The drawing under review shows one solid part. Ordinate dimensions are in mm from its lowest x, y, z. Coordinates: 2 decimals unless noted, no trailing zeros. Loops run counter-clockwise (first coordinate to the right, second up) from the corner with the lowest first, then second, coordinate; pieces in that order, holes last.
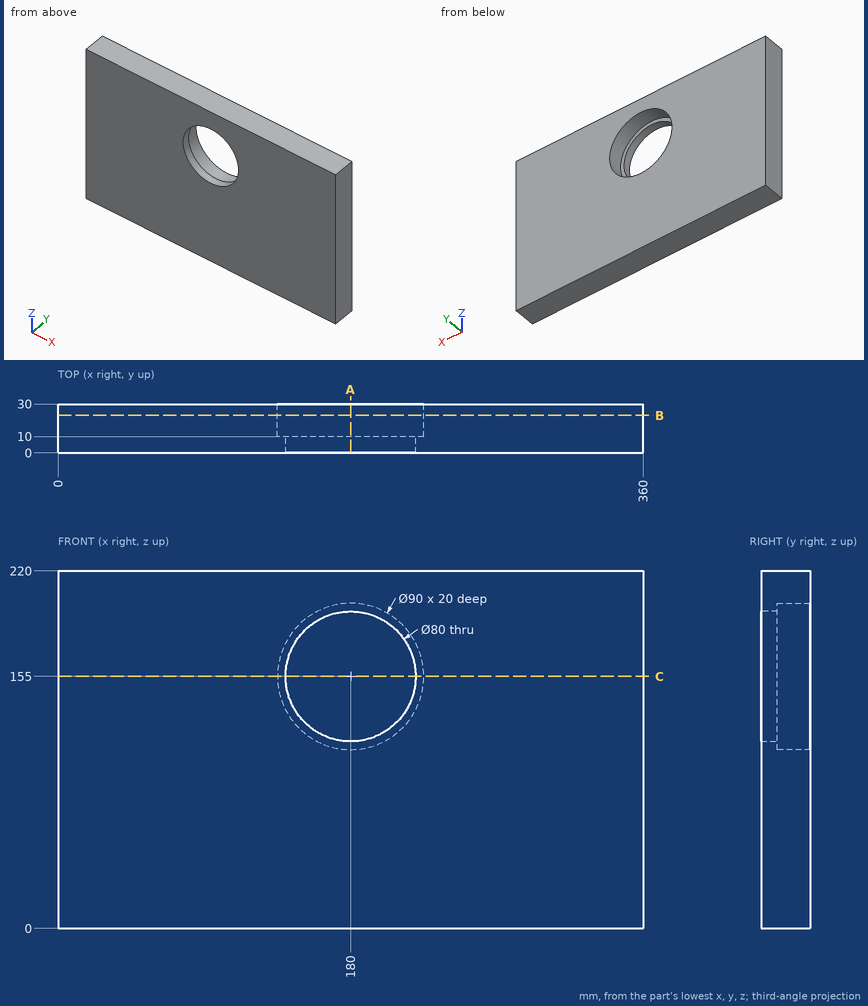
Q1. Take a section at C-C, the plane z = 155. Write out the cut boundary in (x, y).
Q2. Take a section at A-A, the plane x = 180. Write out the cut boundary in (y, z), then the cut area to 3 significant figures.
Q3. Take a section at B-B, the plane y = 23. Write out the cut boundary in (x, z).
Q4. For line 1 (X direction, y = 7.5, z = 155); line 2 (Z direction, x = 154.5, y = 16.25); line 3 (X direction, y = 23.75, z = 155), list the stretches that pass through material, from the lowest coordinate up.
Entries:
1. outline: (0, 0) - (140, 0) - (140, 10) - (135, 10) - (135, 30) - (0, 30) - close; (220, 0) - (360, 0) - (360, 30) - (225, 30) - (225, 10) - (220, 10) - close
2. outline: (0, 0) - (30, 0) - (30, 110) - (10, 110) - (10, 115) - (0, 115) - close; (0, 195) - (10, 195) - (10, 200) - (30, 200) - (30, 220) - (0, 220) - close
2. area: 4,000 mm2
3. outline: (0, 0) - (360, 0) - (360, 220) - (0, 220) - close; hole circle Ø90 at (180, 155)
4. line 1: x = 0 to 140, 220 to 360
4. line 2: z = 0 to 117.92, 192.08 to 220
4. line 3: x = 0 to 135, 225 to 360
